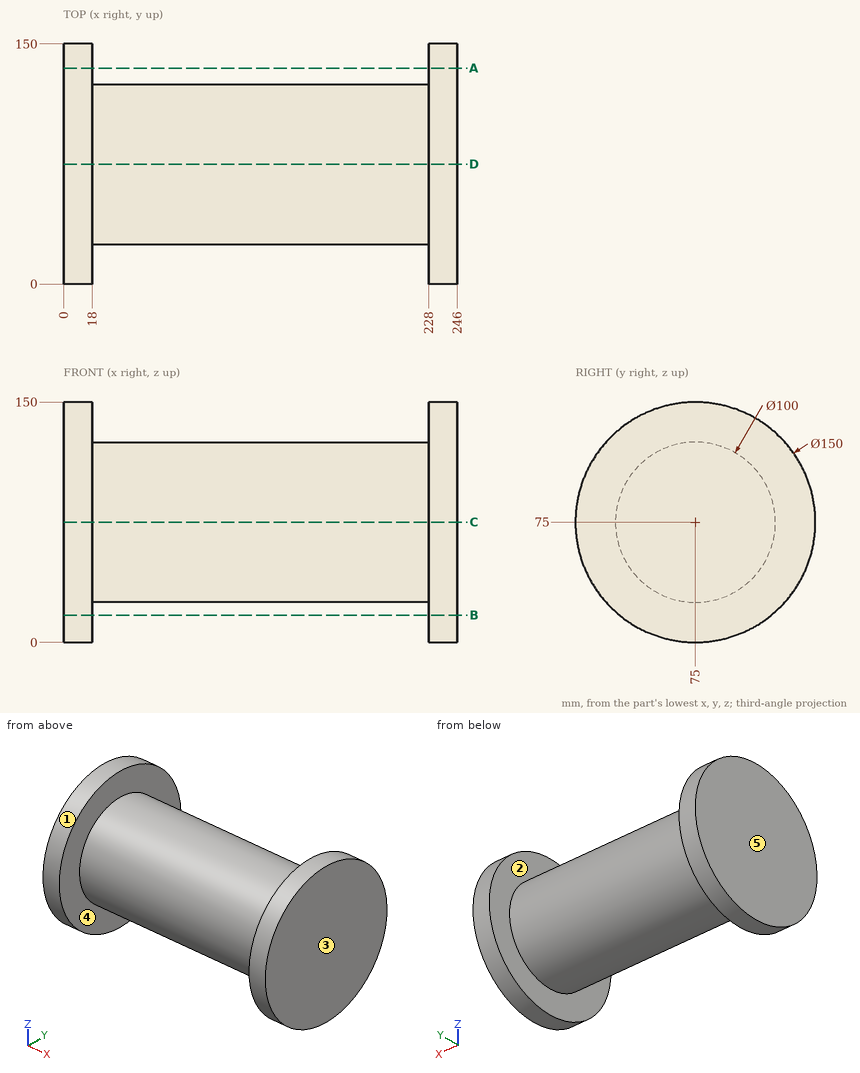
Design review of the part shown in the three views and the two pictorial views. Dimensions are in mm from the part's minimum x, y and z. A direction names the side the tool comes from. Coordinates: 2 decimals unless noted, no trailing zeros. Loops run counter-clockwise (first coordinate to the right, second up) from the corner with the lowest first, then second, coordinate; pieces in that order, holes last. Notation, with made-up numbers: (27, 50) - (76, 50) arc R28 cw to (76, 74) - close; hole circle Ø8 at (15.25, -22). An arc over 180 degrees is marked (long way). Use a Markdown table: item, result. Add a question column.
Item 1: We need section B-B (z = 17). Give the boundary of the cut face in (x, y), and give its area (3 significant figures).
Item 2: We need section A-A (y = 135). Give the boundary of the cut face in (x, z), and give its area (3 significant figures).
Item 3: For line 1 (X direction, y = 134, z = 60); line 2 (Z direction, x = 127, y = 96.5); line 3 (Z direction, x = 42.5, y = 46), list the stretches that pass through material, from the lowest coordinate up.
Item 4: Insertion check: pin 1 Ø4 at (x, y) = (171.5, 83) entering from -Z; pin 2 Ø3 at (x, y) = (148, 64) entering from -Z; pin 3 Ø1 at (x, y) = (47.5, 80) entering from -Z. Each pin has a flat end and moves straight along its axis. Give the tip position at first contact, or say it passes through.
Item 5: We need section C-C (z = 75). Give the boundary of the cut face in (x, y), and give its area (3 significant figures).
Item 6: Mouldability with a two-part tool opening along X and no side actions: class the marked faces 3, 4 and 5 as pulls with the +X half, pulls with the -X half, needs draft (parallel to the pull), parting line crosses it, or undercut.
Item 7: Tool access review of the marked faces 1 and 2: name each direction out of +Z, -Z, +X, -X, +Y, -Y from which nothing blocks a thin tool from reaching the whole face with its end or side.
Results list:
| question | item | result |
|---|---|---|
| 1 | outline | (0, 27.45) - (18, 27.45) - (18, 122.55) - (0, 122.55) - close; (228, 27.45) - (246, 27.45) - (246, 122.55) - (228, 122.55) - close |
| 1 | area | 3,420 mm^2 |
| 2 | outline | (0, 30) - (18, 30) - (18, 120) - (0, 120) - close; (228, 30) - (246, 30) - (246, 120) - (228, 120) - close |
| 2 | area | 3,240 mm^2 |
| 3 | line 1 | x = 0 to 18, 228 to 246 |
| 3 | line 2 | z = 29.86 to 120.14 |
| 3 | line 3 | z = 34.27 to 115.73 |
| 4 | pin 1 | stops at z = 25.36 |
| 4 | pin 2 | stops at z = 25.91 |
| 4 | pin 3 | stops at z = 25.2 |
| 5 | outline | (0, 0) - (18, 0) - (18, 25) - (228, 25) - (228, 0) - (246, 0) - (246, 150) - (228, 150) - (228, 125) - (18, 125) - (18, 150) - (0, 150) - close |
| 5 | area | 26,400 mm^2 |
| 6 | face 3 | pulls with the +X half |
| 6 | face 4 | undercut |
| 6 | face 5 | pulls with the -X half |
| 7 | face 1 | +X, -X |
| 7 | face 2 | none |
